Verification items for the finished model (mm, model axes). A direction names the side the tool comes from. Round coordinates to 2 decimals unless told otherwise and drop trailing zeros. Write each loop counter-clockwise with the first axis right and the second up, starting at its lowest first coordinate (ties: lowest second). Pieces come first, ordered by that corner, then holes. Notation, with made-up numbers: (21.25, 41.5) - (74.25, 41.5) arc R27 cw to (74.25, 66.5) - close; hole circle Ø3 at (-0.75, 9.25). An arc over 180 degrees is marked (long way). Answer as a JSON object with one key per item and string values.
```python
from build123d import *

# Parameters (mm, degrees)
SKETCH_1_R          = 9
EXTRUDE_1_DEPTH     = 14
HOLE_WIZARD_M12_1_D = 10.2


with BuildPart() as part:
    # 草图1 → 凸台-拉伸1 (new body)
    with BuildSketch(Plane.XY):
        Polygon((115, 700), (115, 630), (0, 630), (0, 0), (600, 0), (600, 630), (485, 630), (485, 700), align=None)
        with Locations((440, 470)):
            Circle(SKETCH_1_R, mode=Mode.SUBTRACT)
        with Locations((240, 470)):
            Circle(SKETCH_1_R, mode=Mode.SUBTRACT)
    extrude(amount=EXTRUDE_1_DEPTH)

    # M12 螺纹孔1 (through all)
    with Locations(Plane(origin=(18, 150, 14), x_dir=(1, 0, 0), z_dir=(0, 0, 1))):
        with Locations((0, 0), (90, 0), (0, -90), (90, -90), (474, 130), (564, 130), (474, 40), (564, 40), (222, 160), (362, 160), (222, 20), (362, 20), (222, -120), (362, -120)):
            Hole(HOLE_WIZARD_M12_1_D / 2)


solid = part.part
```
Q1. Release check for a two-part mould opening along Y. For faces 4 (the flat face through (296, 0, 7)), 5 (the cylindrical face through (238.049, 461.214, 6.902)), 6 (the flat face through (600, 311, 7)), 7 (the flat face through (543, 630, 7)) record: released by +Y, released by -Y, zero draft, split by the parting line, or undercut.
Geometry check:
{"face 4": "released by -Y", "face 5": "undercut", "face 6": "zero draft", "face 7": "released by +Y"}
Q2. Section check C-C, the plane x = 558.5. Record the cut outline in (y, z), then the cut area to 3 significant figures.
Geometry check:
{"outline": "(0, 0) - (630, 0) - (630, 14) - (0, 14) - close", "area": "8,820 mm2"}
Q3. Section check B-B, the plane y = 470. Record the cut outline in (x, z), then the cut area to 3 significant figures.
Geometry check:
{"outline": "(0, 0) - (231, 0) - (231, 14) - (0, 14) - close; (249, 0) - (431, 0) - (431, 14) - (249, 14) - close; (449, 0) - (600, 0) - (600, 14) - (449, 14) - close", "area": "7,900 mm2"}
Q4. Material ranges on line 1 along Y through (x, z) = (240, 10.75); line 2 along Y through (x, z) = (582, 3); line 3 along X through (y, z) = (149, 6.5), recorded low to high. Write a range as [from, to].
Geometry check:
{"line 1": "y = [0, 24.9], [35.1, 164.9], [175.1, 304.9], [315.1, 461], [479, 700]", "line 2": "y = [0, 184.9], [195.1, 274.9], [285.1, 630]", "line 3": "x = [0, 13], [23, 103], [113, 600]"}
Q5. Gauge pin test, flat ends, axial feed: P1, Ø6, axis at x = 87.5, z = 4, coming from the +Y side; P2, Ø8, axis at x = 108, y = 150, coming from the +Z side. Record the tip position at first contact, or that the pin passes through.
Geometry check:
{"P1": "stops at y = 630", "P2": "passes through"}
Q6. Section check A-A, the plane z = 5.5. State how many separate pieces and enclosed holes the cut face has, then the cut area to 3 significant figures.
Geometry check:
{"separate pieces": "1", "enclosed holes": "16", "area": "402,000 mm2"}
Q7. Set-up check for faces 1 (the flat face through (296, 355, 14)), 2 (the flat face through (485, 665, 7)), 3 (the flat face through (115, 665, 7)): record each of +Z, -Z, +X, -X, +Y, -Y from which the full face is reachable in a straight line by a thin tool's end or side.
Geometry check:
{"face 1": "+Z, +X, -X, +Y, -Y", "face 2": "+Z, -Z, +X, +Y", "face 3": "+Z, -Z, -X, +Y"}
